Work out the finished part from the listing and answer in its coordinate system (mm). A direction names the side the tool comes from. Coordinates: 2 decimals unless noted, no trailing zeros. Order: outer loops, then holes, each group sorted by start corner. A loop starts at its lowest first (then second) coordinate and runs counter-clockwise, first axis right, second up. Notation, with made-up numbers: M 69.5,-27.75 L 76.5,-27.75 A12 cw 76.5,-23.75 Z; hole C -0.5,68.5 d1. An arc over 180 degrees is marked long. Use a Markdown table: item, result. Add a question column.
from build123d import *

# Parameters (mm, degrees)
BOSS_EXTRUDE1_DEPTH = 20
CHAMFER1_SIZE       = 12


with BuildPart() as part:
    # Sketch1 → Boss-Extrude1 (new, symmetric)
    with BuildSketch(Plane(origin=(0, 0, 0), x_dir=(0, 0, -1), z_dir=(1, 0, 0))):
        Polygon((0, 0), (70, -35), (70, 194), (0, 194), align=None)
        with BuildLine():
            Line((32.5, 114), (32.5, 164))
            ThreePointArc((32.5, 164), (45, 176.5), (57.5, 164))
            Line((57.5, 164), (57.5, 114))
            ThreePointArc((57.5, 114), (45, 101.5), (32.5, 114))
        make_face(mode=Mode.SUBTRACT)
        with BuildLine():
            Line((32.5, 30.910324642), (32.5, 64))
            ThreePointArc((32.5, 64), (45, 76.5), (57.5, 64))
            Line((57.5, 64), (57.5, 30.910324642))
            ThreePointArc((57.5, 30.910324642), (45, 18.410324642), (32.5, 30.910324642))
        make_face(mode=Mode.SUBTRACT)
    extrude(amount=BOSS_EXTRUDE1_DEPTH, both=True)

    # Chamfer1
    chamfer1_edges = [part.edges().sort_by_distance(p)[0] for p in [
        (-20, 194, -35),
        (-20, 79.5, -70),
        (-20, -17.5, -35),
        (-20, 97, 0),
    ]]
    chamfer(chamfer1_edges, length=CHAMFER1_SIZE)


solid = part.part
(1) A cutting plane is placed at C-C on z = -52. Write down the section's boundary in (x, y).
(2) A cutting plane is placed at A-A on y = 120. Write down the section's boundary in (x, z), plus the area to 3 significant figures.
(3) A cutting plane is placed at B-B on x = -4. Write down the section's boundary in (y, z).
(4) Which of the six approach directions +Z, -Z, +X, -X, +Y, -Y give full straight-line access (tool end or side, diameter ignored) to faces 4 (the flat face through (20, 81, -35)), 5 (the cylindrical face through (0.28, 101.503, -45.275))?
(5) A cutting plane is placed at D-D on y = 14. Write down the section's boundary in (x, z).
(6) The mould has two halves that part along Z. Classify faces 1 (the flat face through (-14.084, -11.813, -37.231)), 2 (the flat face through (0, 48, -57.5)), 3 (the flat face through (6, 78, -70)): pulls with the +Z half, pulls with the -Z half, needs draft (parallel to the pull), parting line crosses it, or undercut.
(7) Straight lines are drawn through the part: line 1 (Z direction, x = 15, y = 131.5); line 2 (Y direction, x = -3, z = -48); line 3 (Y direction, x = 1, z = -39.5). For each, find the intervals that lie inside material, in ascending order.
(8) Given P1, Ø5, axis at x = 10.5, z = -41, coming from the -Y side; P2, Ø12, axis at x = 1, z = -24, coming from the -Y side, each flat-ended and moving along its own axis, determine where each tip first touches the part or whether it passes through.
From the geometry:
| question | item | result |
|---|---|---|
| 1 | outline | M -20,-12.58 L -8,-26 L 20,-26 L 20,20.55 L -20,20.55 Z; M -20,74.36 L 20,74.36 L 20,103.64 L -20,103.64 Z; M -20,174.36 L 20,174.36 L 20,194 L -8,194 L -20,182 Z |
| 2 | outline | M -20,-58 L -8,-70 L 20,-70 L 20,-57.5 L -20,-57.5 Z; M -20,-32.5 L 20,-32.5 L 20,0 L -8,0 L -20,-12 Z |
| 2 | area | 1,660 mm2 |
| 3 | outline | M -35,-70 L 194,-70 L 194,0 L 0,0 Z; hole M 30.91,-57.5 L 64,-57.5 A12.5 ccw 64,-32.5 L 30.91,-32.5 A12.5 ccw Z; hole M 114,-57.5 L 164,-57.5 A12.5 ccw 164,-32.5 L 114,-32.5 A12.5 ccw Z |
| 4 | face 4 | +Z, -Z, +X, +Y, -Y |
| 4 | face 5 | +X, -X |
| 5 | outline | M -20,-58 L -8,-70 L 20,-70 L 20,0 L -8,0 L -20,-12 Z |
| 6 | face 1 | pulls with the +Z half |
| 6 | face 2 | undercut |
| 6 | face 3 | pulls with the -Z half |
| 7 | line 1 | z = -70 to -57.5, -32.5 to 0 |
| 7 | line 2 | y = -24 to 18.78, 76.13 to 101.87, 176.13 to 194 |
| 7 | line 3 | y = -19.75 to 19.69, 75.22 to 102.78, 175.22 to 194 |
| 8 | P1 | stops at y = -21.75 |
| 8 | P2 | stops at y = -15 |
